```python
from build123d import *

# Parameters (mm, degrees)
SKETCH1_R           = 5
SKETCH1_R_2         = 1.9
BOSS_EXTRUDE1_DEPTH = 0.5


with BuildPart() as part:
    # Sketch1 → Boss-Extrude1 (new body)
    with BuildSketch(Plane.XY):
        with BuildLine():
            ThreePointArc((-11.621881793, 4.602375864), (-12.5, 0), (-11.621881793, -4.602375864))
            ThreePointArc((-11.621881793, -4.602375864), (-10.835386311, -5.223871597), (-9.904943546, -4.850899277))
            ThreePointArc((-9.904943546, -4.850899277), (-4.5254834, -4.5254834), (-4.850899277, -9.904943546))
            ThreePointArc((-4.850899277, -9.904943546), (-5.223871597, -10.835386311), (-4.602375864, -11.621881793))
            ThreePointArc((-4.602375864, -11.621881793), (0, -12.5), (4.602375864, -11.621881793))
            ThreePointArc((4.602375864, -11.621881793), (5.223871597, -10.835386311), (4.850899277, -9.904943546))
            ThreePointArc((4.850899277, -9.904943546), (4.5254834, -4.5254834), (9.904943546, -4.850899277))
            ThreePointArc((9.904943546, -4.850899277), (10.835386311, -5.223871597), (11.621881793, -4.602375864))
            ThreePointArc((11.621881793, -4.602375864), (12.5, 0), (11.621881793, 4.602375864))
            ThreePointArc((11.621881793, 4.602375864), (10.835386311, 5.223871597), (9.904943546, 4.850899277))
            ThreePointArc((9.904943546, 4.850899277), (4.5254834, 4.5254834), (4.850899277, 9.904943546))
            ThreePointArc((4.850899277, 9.904943546), (5.223871597, 10.835386311), (4.602375864, 11.621881793))
            ThreePointArc((4.602375864, 11.621881793), (0, 12.5), (-4.602375864, 11.621881793))
            ThreePointArc((-4.602375864, 11.621881793), (-5.223871597, 10.835386311), (-4.850899277, 9.904943546))
            ThreePointArc((-4.850899277, 9.904943546), (-4.5254834, 4.5254834), (-9.904943546, 4.850899277))
            ThreePointArc((-9.904943546, 4.850899277), (-10.835386311, 5.223871597), (-11.621881793, 4.602375864))
        make_face()
        Circle(SKETCH1_R, mode=Mode.SUBTRACT)
        with Locations((0, 9.5)):
            Circle(SKETCH1_R_2, mode=Mode.SUBTRACT)
        with Locations((9.5, 0)):
            Circle(SKETCH1_R_2, mode=Mode.SUBTRACT)
        with Locations((0, -9.5)):
            Circle(SKETCH1_R_2, mode=Mode.SUBTRACT)
        with Locations((-9.5, 0)):
            Circle(SKETCH1_R_2, mode=Mode.SUBTRACT)
    extrude(amount=BOSS_EXTRUDE1_DEPTH)


solid = part.part
```
CAD build for the part. Positions are in the model's coordinates, mm. Round coordinates to 2 decimals unless told otherwise and drop trailing zeros. Order: outer loops, then holes, each group sorted by start corner. A loop starts at its lowest first (then second) coordinate and runs counter-clockwise, first axis right, second up.
Q1. Slice it at A-A (y = 0). Write the cut outline in (x, z), and give its area (3 significant figures).
Q2. Drop flat-ended pins along their axis: pin 1 (6.5 mm diameter, centred on x = -7.07, y = -7.07, fed in from -Z); pin 2 (9.5 mm diameter, centred on x = 7.07, y = -7.07, fed in from -Z). Give the stop position or say it passes through.
Q3. Slice it at D-D (x = 9.5). Write the cut outline in (y, z).
Q4. Wall check: L1, parallel to Y at x = 0, z = 0.45; L2, parallel to Y at x = -1.5, z = 0.2; L3, parallel to X at y = 0.25, z = 0.15. Give the ranges that are in metal, low to high.
Q5. Slice it at C-C (y = 10.75). Write the cut outline in (x, z), and give its area (3 significant figures).
Q6. Two-plate mould, pull along X, no slides. Class faces 1 (the cylindrical face through (0.877, -11.186, 0.246)), 2 (the cylindrical face through (-0.1, -12.5, 0.2)), 3 (the cylindrical face through (-12.5, 0.1, 0.2)): pulls with the +X half, pulls with the -X half, needs draft (parallel to the pull), parting line crosses it, or undercut.
Results below:
1. outline: (-12.5, 0) - (-11.4, 0) - (-11.4, 0.5) - (-12.5, 0.5) - close; (-7.6, 0) - (-5, 0) - (-5, 0.5) - (-7.6, 0.5) - close; (5, 0) - (7.6, 0) - (7.6, 0.5) - (5, 0.5) - close; (11.4, 0) - (12.5, 0) - (12.5, 0.5) - (11.4, 0.5) - close
1. area: 3.70 mm2
2. pin 1: passes through
2. pin 2: stops at z = 0
3. outline: (-4.41, 0) - (-1.9, 0) - (-1.9, 0.5) - (-4.41, 0.5) - close; (1.9, 0) - (4.41, 0) - (4.41, 0.5) - (1.9, 0.5) - close
4. L1: y = -12.5 to -11.4, -7.6 to -5, 5 to 7.6, 11.4 to 12.5
4. L2: y = -12.41 to -10.67, -8.33 to -4.77, 4.77 to 8.33, 10.67 to 12.41
4. L3: x = -12.5 to -11.38, -7.62 to -4.99, 4.99 to 7.62, 11.38 to 12.5
5. outline: (-5.23, 0) - (-1.43, 0) - (-1.43, 0.5) - (-5.23, 0.5) - close; (1.43, 0) - (5.23, 0) - (5.23, 0.5) - (1.43, 0.5) - close
5. area: 3.80 mm2
6. face 1: undercut
6. face 2: parting line crosses it
6. face 3: pulls with the -X half
